Design review of the part shown in the three views and the two pictorial views. Dimensions are in mm from the part's minimum x, y and z. Round coordinates to 2 decimals unless told otherwise and drop trailing zeros. Write each loop counter-clockwise with the first axis right and the second up, starting at its lowest first coordinate (ties: lowest second). Pieces come first, ordered by that corner, then holes. Notation, with made-up numbers: (-21.75, -10) -> (-3.75, -10) arc R20 ccw to (-3.75, 26) -> close; hole circle Ø3 at (3, 58). An arc over 180 degrees is marked (long way). Answer as a JSON object with one key per item and string values. Group by question number.
1) We need section B-B, the plane z = 4. Write out the cut boundary in (x, y).
2) We need section A-A, the plane y = 20. Write out the cut boundary in (x, z), then the cut area to 3 significant figures.
3) We need section C-C, the plane x = 85. Write out the cut boundary in (y, z), then the cut area to 3 significant figures.
4) To check wall thickness, follow probe 1 along Y at (x, z) = (30, 10.75); probe 2 along Y at (x, z) = (88.5, 2.5); probe 3 along X at (y, z) = (83, 3.25). State the ranges of each line that lie inside material, in increasing order. Write a range as [from, to].
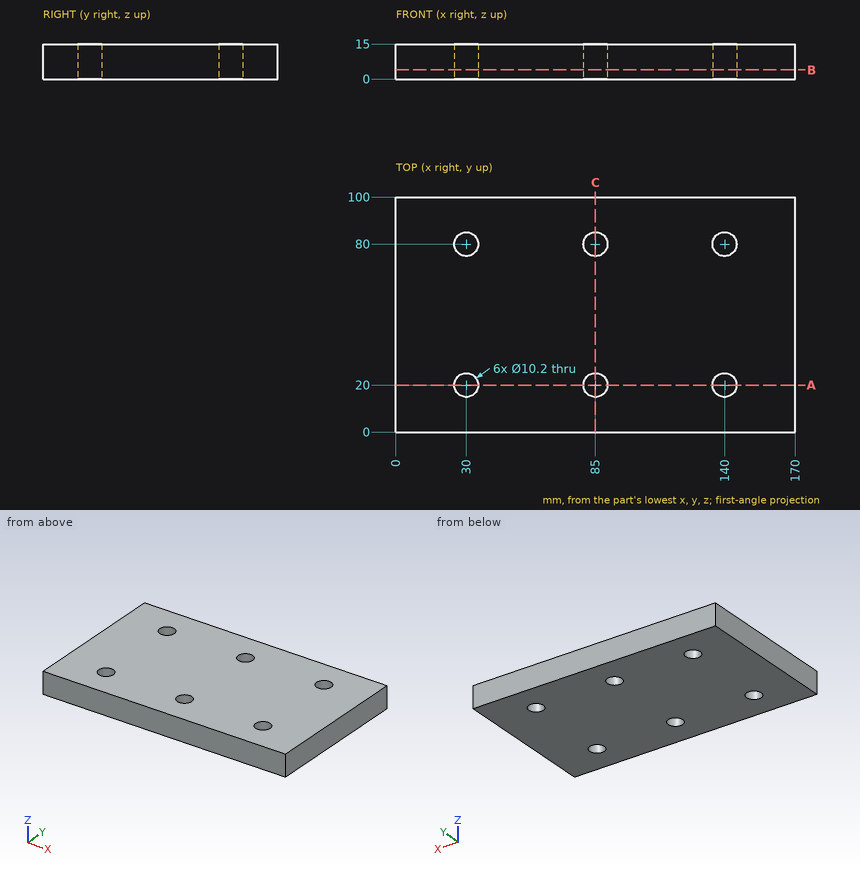
Here are the results:
{
 "1": {"outline": "(0, 0) -> (170, 0) -> (170, 100) -> (0, 100) -> close; hole circle Ø10.2 at (30, 20); hole circle Ø10.2 at (30, 80); hole circle Ø10.2 at (85, 20); hole circle Ø10.2 at (85, 80); hole circle Ø10.2 at (140, 20); hole circle Ø10.2 at (140, 80)"},
 "2": {"outline": "(0, 0) -> (24.9, 0) -> (24.9, 15) -> (0, 15) -> close; (35.1, 0) -> (79.9, 0) -> (79.9, 15) -> (35.1, 15) -> close; (90.1, 0) -> (134.9, 0) -> (134.9, 15) -> (90.1, 15) -> close; (145.1, 0) -> (170, 0) -> (170, 15) -> (145.1, 15) -> close", "area": "2,090 mm^2"},
 "3": {"outline": "(0, 0) -> (14.9, 0) -> (14.9, 15) -> (0, 15) -> close; (25.1, 0) -> (74.9, 0) -> (74.9, 15) -> (25.1, 15) -> close; (85.1, 0) -> (100, 0) -> (100, 15) -> (85.1, 15) -> close", "area": "1,190 mm^2"},
 "4": {"probe 1": "y = [0, 14.9], [25.1, 74.9], [85.1, 100]", "probe 2": "y = [0, 16.29], [23.71, 76.29], [83.71, 100]", "probe 3": "x = [0, 25.88], [34.12, 80.88], [89.12, 135.88], [144.12, 170]"}
}
